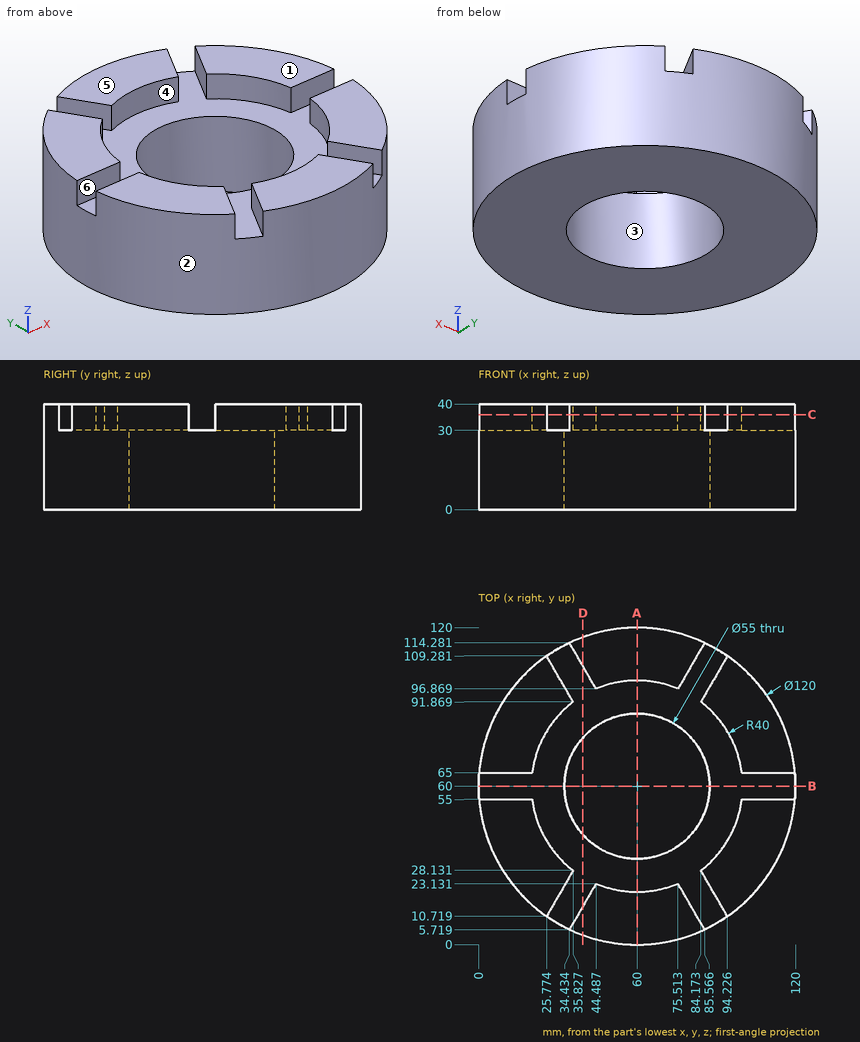
The figure shows three views and two pictorial views of one solid part (mm, origin at its lowest corner). Answer the questions. A direction names the side the tool comes from. Coordinates: 2 decimals unless noted, no trailing zeros. Loops run counter-clockwise (first coordinate to the right, second up) from the corner with the lowest first, then second, coordinate; pieces in that order, holes last. Notation, with made-up numbers: (75.5, -38) -> (118.5, -38) arc R24 cw to (118.5, -2) -> close; hole circle Ø4 at (-21.5, 45). An arc over 180 degrees is marked (long way). Return JSON: item names as keys, results as strings. Group by question number.
(1) Given pin 1 Ø1 at (x, z) = (13, 25) entering from +Y; pin 2 Ø6 at (y, z) = (102.5, 17) entering from +X (1 decimal); pin 3 Ø8 at (x, z) = (29, 26.5) entering from -Y, each flat-ended and moving along its own axis, determine where each tip first touches the part or whether it passes through.
(2) Which of the six approach directions +Z, -Z, +X, -X, +Y, -Y give full straight-line access (tool end or side, diameter ignored) to the marked faces 4, 5 and 6?
(3) A cutting plane is placed at C-C on z = 36. Write down the section's boundary in (x, y) (1 decimal).
(4) A cutting plane is placed at D-D on x = 39.5. Write down the section's boundary in (y, z).
(5) Find the intervals of material crossed by probe 1 along Y at (x, z) = (60, 7); probe 2 along Z at (x, y) = (41.5, 100); probe 3 along X at (y, z) = (59, 20), in increasing order. Write a range as from..to.
(6) A cutting plane is placed at A-A on x = 60. Write down the section's boundary in (y, z), and give its area (3 significant figures).
(7) A cutting plane is placed at B-B on y = 60. Write down the section's boundary in (x, z), and give its area (3 significant figures).
(8) Determine the mould class of the marked faces 1, 2 and 3 for opening direction Y: released by +Y, released by -Y, zero draft, split by the parting line, or undercut.
The answers:
{
 "1": {"pin 1": "stops at y = 97.92", "pin 2": "stops at x = 105.2", "pin 3": "stops at y = 6.42"},
 "2": {"face 4": "+Z", "face 5": "+Z, +X, -X, +Y, -Y", "face 6": "+Z, +X, -X"},
 "3": {"outline": "(0.2, 55) arc R60 ccw to (25.8, 10.7) -> (35.8, 28.1) arc R40 cw to (20.3, 55) -> close; (0.2, 65) -> (20.3, 65) arc R40 cw to (35.8, 91.9) -> (25.8, 109.3) arc R60 ccw to start; (34.4, 5.7) arc R60 ccw to (85.6, 5.7) -> (75.5, 23.1) arc R40 cw to (44.5, 23.1) -> close; (34.4, 114.3) -> (44.5, 96.9) arc R40 cw to (75.5, 96.9) -> (85.6, 114.3) arc R60 ccw to start; (84.2, 28.1) -> (94.2, 10.7) arc R60 ccw to (119.8, 55) -> (99.7, 55) arc R40 cw to start; (84.2, 91.9) arc R40 cw to (99.7, 65) -> (119.8, 65) arc R60 ccw to (94.2, 109.3) -> close"},
 "4": {"outline": "(3.61, 0) -> (41.67, 0) -> (41.67, 30) -> (14.49, 30) -> (14.49, 40) -> (3.61, 40) -> close; (78.33, 0) -> (116.39, 0) -> (116.39, 40) -> (105.51, 40) -> (105.51, 30) -> (78.33, 30) -> close"},
 "5": {"probe 1": "y = 0..32.5, 87.5..120", "probe 2": "z = 0..30", "probe 3": "x = 0.01..32.52, 87.48..119.99"},
 "6": {"outline": "(0, 0) -> (32.5, 0) -> (32.5, 30) -> (20, 30) -> (20, 40) -> (0, 40) -> close; (87.5, 0) -> (120, 0) -> (120, 40) -> (100, 40) -> (100, 30) -> (87.5, 30) -> close", "area": "2,350 mm^2"},
 "7": {"outline": "(0, 0) -> (32.5, 0) -> (32.5, 30) -> (0, 30) -> close; (87.5, 0) -> (120, 0) -> (120, 30) -> (87.5, 30) -> close", "area": "1,950 mm^2"},
 "8": {"face 1": "zero draft", "face 2": "split by the parting line", "face 3": "undercut"}
}
